```python
from build123d import *

# Parameters (mm, degrees)
BOSS_EXTRUDE1_DEPTH = 5
CHAMFER1_SIZE       = 10


with BuildPart() as part:
    # Sketch1 → Boss-Extrude1 (new, symmetric)
    with BuildSketch(Plane.XY):
        with BuildLine():
            Line((-85, 0), (-80, 0))
            Line((-80, 0), (-43.022132459, 60.231945943))
            ThreePointArc((-43.022132459, 60.231945943), (-39.382649924, 63.726954206), (-34.5, 65))
            Line((-34.5, 65), (34.5, 65))
            ThreePointArc((34.5, 65), (39.382649924, 63.726954206), (43.022132459, 60.231945943))
            Line((43.022132459, 60.231945943), (80, 0))
            Line((80, 0), (85, 0))
            Line((85, 0), (85, 75))
            Line((85, 75), (-85, 75))
            Line((-85, 75), (-85, 0))
        make_face()
    extrude(amount=BOSS_EXTRUDE1_DEPTH, both=True)

    # Chamfer1
    chamfer1_edges = [part.edges().sort_by_distance(p)[0] for p in [
        (-85, 75, 0),
        (85, 75, 0),
    ]]
    chamfer(chamfer1_edges, length=CHAMFER1_SIZE)


solid = part.part
```
Part model, mm, in its own coordinate system. A direction names the side the tool comes from. Round coordinates to 2 decimals unless told otherwise and drop trailing zeros. Loops run counter-clockwise (first coordinate to the right, second up) from the corner with the lowest first, then second, coordinate; pieces in that order, holes last.
Item 1: Cut at D-D, the plane x = 1. Give the cut face in (y, z), then the cut area to 3 significant figures.
Item 2: Cut at A-A, the plane y = 63. Give the cut face in (x, z).
Item 3: Cut at C-C, the plane y = 53.5. Give the cut face in (x, z), then the cut area to 3 significant figures.
Item 4: Cut at B-B, the plane z = 2.25. Give the cut face in (x, y).
Item 5: Drop flat-ended pins along their axis: P1, Ø2, axis at x = 68, z = 1, coming from the -Y side; P2, Ø5, axis at y = 67, z = -0.5, coming from the +X side. Give the stop position or say it passes through.
Item 6: Mould opens along X. For faces 3 (the face through (-39.445, 63.692, 0.07)), 4 (the face through (1, 75, 0)), 5 (the face through (85, 32, 0)) say: +X half, -X half, draft (parallel to the pull), parting line (faces both ways), or undercut.
Item 7: Drill centre lines: line 1 (X direction, y = 20, z = -3); line 2 (Y direction, x = 3.5, z = 2.75); line 3 (X direction, y = 6, z = -1.5). Where is each one in solid material? Low to high.
Item 8: 3-axis set-ups, long thin cutter, end or side, ignore diameter. For faces 1 (the face through (0, 65, 0)), 2 (the face through (-85, 33, 0)): which of +Z, -Z, +X, -X, +Y, -Y reach the whole face in a straight line?
A:
1. outline: (65, -5) - (75, -5) - (75, 5) - (65, 5) - close
1. area: 100 mm2
2. outline: (-85, -5) - (-40.5, -5) - (-40.5, 5) - (-85, 5) - close; (40.5, -5) - (85, -5) - (85, 5) - (40.5, 5) - close
3. outline: (-85, -5) - (-47.16, -5) - (-47.16, 5) - (-85, 5) - close; (47.16, -5) - (85, -5) - (85, 5) - (47.16, 5) - close
3. area: 757 mm2
4. outline: (-85, 0) - (-80, 0) - (-43.02, 60.23) arc R10 cw to (-34.5, 65) - (34.5, 65) arc R10 cw to (43.02, 60.23) - (80, 0) - (85, 0) - (85, 65) - (75, 75) - (-75, 75) - (-85, 65) - close
5. P1: stops at y = 17.92
5. P2: stops at x = 85
6. face 3: undercut
6. face 4: draft
6. face 5: +X half
7. line 1: x = -85 to -67.72, 67.72 to 85
7. line 2: y = 65 to 75
7. line 3: x = -85 to -76.32, 76.32 to 85
8. face 1: +Z, -Z, -Y
8. face 2: +Z, -Z, -X, +Y, -Y
